Input: dimensioned drawing with shaded views. Units: mm. Origin: part minimum x, y, z. A direction names the side the tool comes from. Coordinates: 2 decimals unless noted, no trailing zeros. Loops run counter-clockwise (first coordinate to the right, second up) from the corner with the lowest first, then second, coordinate; pieces in that order, holes last.
Item 1: Section D-D on x = 13.75. Return loops of the section in (y, z).
Item 2: Contact query for flat-ended pins moving along their axis: P1, Ø5, axis at x = 22, y = 4.5, coming from the -Z side; P2, Ø6, axis at x = 11, z = 20, coming from the -Y side; P3, Ø1.5, axis at x = 3.5, z = 9.5, coming from the +Y side. Output: stop coordinate, or through.
Item 3: Section B-B on y = 5.75. Return loops of the section in (x, z).
Item 4: Ray query, line 1 along X through (y, z) = (4.75, 24.5); line 2 along Z through (x, y) = (23.5, 4.5); line 3 along X through (y, z) = (8, 24.5). Return the intervals inside material, ascending.
Item 5: Section A-A on y = 3.25. Return loops of the section in (x, z), and give its area (3 significant figures).
Item 6: Reachability of the marked faces 1 and 2 from +Z, -Z, +X, -X, +Y, -Y: full face, straight path, thin tool, end or side. Return the list, or none.
Item 7: Section C-C on z = 5.5. Return loops of the section in (x, y), and give its area (3 significant figures).
Item 8: Pull-direction query (X, two-part tool) for the marked faces 3, 4, 5 and 6; classes: released by +X, released by -X, zero draft, split by the parting line, or undercut.
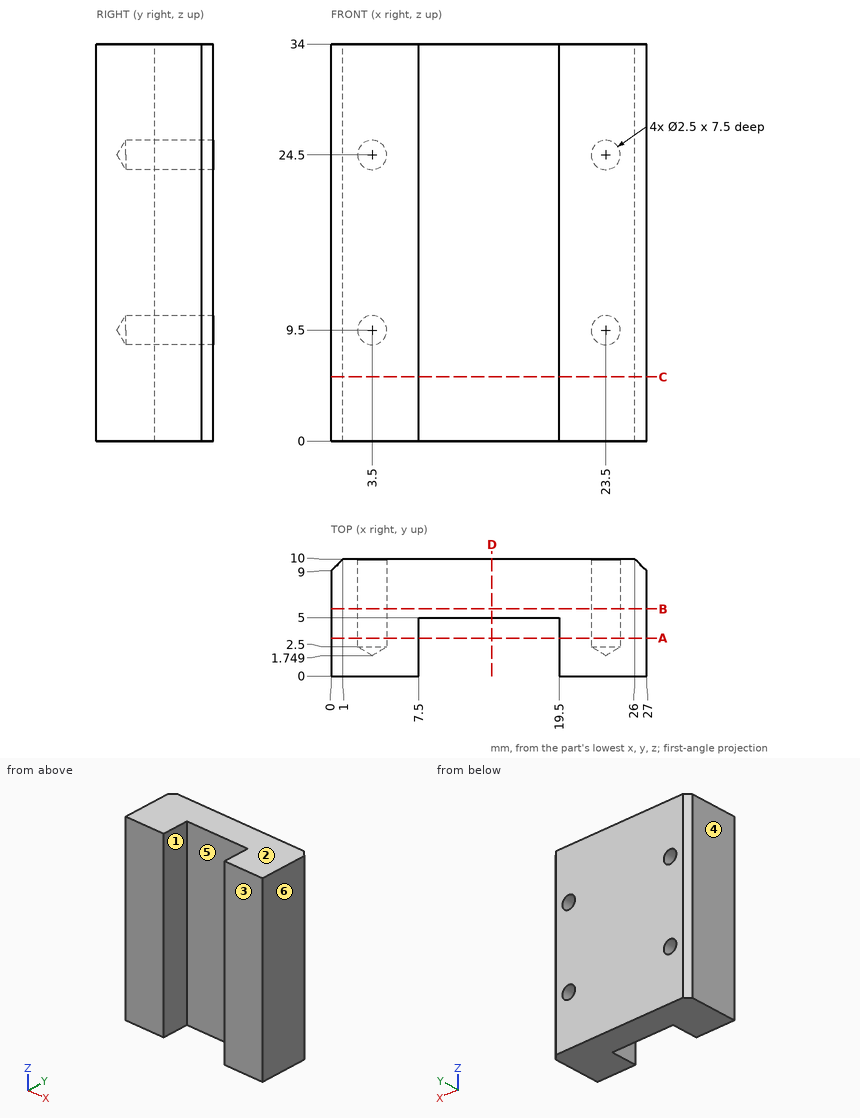
Results found:
1. outline: (5, 0) - (10, 0) - (10, 34) - (5, 34) - close
2. P1: stops at z = 0
2. P2: stops at y = 5
2. P3: stops at y = 2.2
3. outline: (0, 0) - (27, 0) - (27, 34) - (0, 34) - close; hole circle Ø2.5 at (3.5, 9.5); hole circle Ø2.5 at (3.5, 24.5); hole circle Ø2.5 at (23.5, 9.5); hole circle Ø2.5 at (23.5, 24.5)
4. line 1: x = 0 to 2.25, 4.75 to 7.5, 19.5 to 22.25, 24.75 to 27
4. line 2: z = 0 to 8.25, 10.75 to 23.25, 25.75 to 34
4. line 3: x = 0 to 2.25, 4.75 to 22.25, 24.75 to 27
5. outline: (0, 0) - (7.5, 0) - (7.5, 34) - (0, 34) - close; (19.5, 0) - (27, 0) - (27, 34) - (19.5, 34) - close; hole circle Ø2.5 at (3.5, 9.5); hole circle Ø2.5 at (3.5, 24.5); hole circle Ø2.5 at (23.5, 9.5); hole circle Ø2.5 at (23.5, 24.5)
5. area: 490 mm2
6. face 1: +Z, -Z, -Y
6. face 2: +Z, +X, -X, +Y, -Y
7. outline: (0, 0) - (7.5, 0) - (7.5, 5) - (19.5, 5) - (19.5, 0) - (27, 0) - (27, 9) - (26, 10) - (1, 10) - (0, 9) - close
7. area: 209 mm2
8. face 3: zero draft
8. face 4: released by -X
8. face 5: undercut
8. face 6: released by +X
